Read the model definition and answer for the solid it produces. Units are mm, in the model's axes. Round coordinates to 2 decimals unless told otherwise and drop trailing zeros.
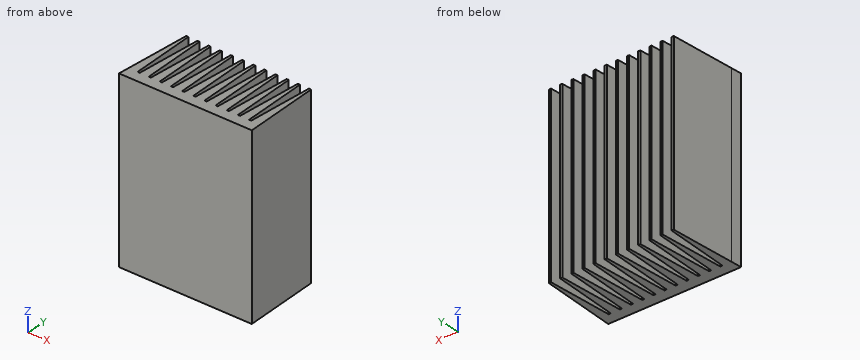
from build123d import *

# Parameters (mm, degrees)
BASE_PROFILE_SKETCH_W      = 61.21
BASE_PROFILE_SKETCH_H      = 80
HEAT_SINK_BASE_BLOCK_DEPTH = 35
FIN_SLOTS_CUT_DEPTH        = 105
SIDE_TRIM_CUT_DEPTH        = 180.145


with BuildPart() as part:
    # Base Profile Sketch → Heat Sink Base Block (new body)
    with BuildSketch(Plane(origin=(0, 0, 0), x_dir=(1, 0, 0), z_dir=(0, 1, 0))):
        with Locations((-0.605, 0)):
            Rectangle(BASE_PROFILE_SKETCH_W, BASE_PROFILE_SKETCH_H)
    extrude(amount=HEAT_SINK_BASE_BLOCK_DEPTH)

    # Fin Slots Sketch → Fin Slots Cut (cut)
    with BuildSketch(Plane.XY.offset(40)):
        Polygon((23.025727725, 35), (24.597961104, 5), (25.593494347, 5), (27.165727725, 35), align=None)
        Polygon((28.165727725, 35), (30, 0), (30, 35), align=None)
        Polygon((20.453494347, 5), (22.025727725, 35), (22.021260968, 35), (17.885727725, 35), (19.457961104, 5), align=None)
        Polygon((15.313494347, 5), (16.885727725, 35), (12.745727725, 35), (14.317961104, 5), align=None)
        Polygon((10.173494347, 5), (11.745727725, 35), (7.605727725, 35), (9.177961104, 5), align=None)
        Polygon((5.033494347, 5), (6.605727725, 35), (2.465727725, 35), (4.037961104, 5), align=None)
        Polygon((-0.106505653, 5), (1.465727725, 35), (-2.674272275, 35), (-1.102038896, 5), align=None)
        Polygon((-5.246505653, 5), (-3.674272275, 35), (-7.814272275, 35), (-6.242038896, 5), align=None)
        Polygon((-10.386505653, 5), (-8.814272275, 35), (-12.954272275, 35), (-11.382038896, 5), align=None)
        Polygon((-15.526505653, 5), (-13.954272275, 35), (-18.094272275, 35), (-16.522038896, 5), align=None)
        Polygon((-20.666505653, 5), (-19.094272275, 35), (-23.234272275, 35), (-21.662038896, 5), align=None)
        Polygon((-25.806505653, 5), (-24.234272275, 35), (-28.374272275, 35), (-26.802038896, 5), align=None)
        Polygon((-30.946505653, 5), (-29.374272275, 35), (-31.20854455, 35), (-31.20854455, 5), align=None)
    extrude(amount=-FIN_SLOTS_CUT_DEPTH, mode=Mode.SUBTRACT)

    # Side Trim Sketch → Side Trim Cut (cut)
    with BuildSketch(Plane.XY.offset(40)):
        Polygon((-29.374272275, 35), (-31.21, 0), (-36.791681348, 0), (-36.791681348, 36.336825614), (-29.374272275, 36.336825614), align=None)
    extrude(amount=-SIDE_TRIM_CUT_DEPTH, mode=Mode.SUBTRACT)


solid = part.part
Q1. A straight line is drawn through the part: probe 1 along Y at (x, z) = (25, 15). Find the intervals that lie inside material, in ascending order.
Outcome:
probe 1: y = 0 to 5
Q2. Flat-ended cylindrical pins translate along their axes: pin 1 (0.5 mm diameter, centred on x = 4.5, z = -6.5, fed in from +Y); pin 2 (5 mm diameter, centred on y = 26.5, z = 1, fed in from +X); pin 3 (1.5 mm diameter, centred on y = 31.5, z = -31, fed in from +X); pin 4 (8 mm diameter, centred on x = -22.5, y = 27.5, fed in from +Z). Find the tip coordinate at first contact, or state that the pin passes through.
Outcome:
pin 1: stops at y = 5
pin 2: stops at x = 28.74
pin 3: stops at x = 28.39
pin 4: stops at z = 40
Q3. A cutting plane is placed at A-A, the plane y = 25. Give the number of separate pieces and of enclosed holes in the cut face, plus the area to 3 significant figures.
Outcome:
separate pieces: 12
enclosed holes: 0
area: 1,970 mm2
